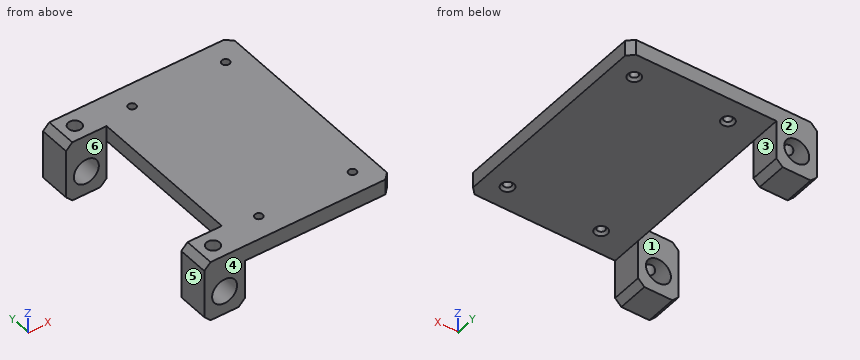
```python
from build123d import *

# Parameters (mm, degrees)
BOSS_EXTRUDE1_DEPTH   = 70
SKETCH2_R             = 0.75
CUT_EXTRUDE1_DEPTH    = 10
SKETCH3_W             = 25
SKETCH3_H             = 50
CUT_EXTRUDE2_DEPTH    = 13
SKETCH4_R             = 4
CUT_EXTRUDE3_DEPTH    = 96.524865873
SKETCH5_W             = 13
SKETCH5_H             = 50
BOSS_EXTRUDE2_DEPTH   = 5
SKETCH9_W             = 13
SKETCH9_H             = 5.5
CUT_EXTRUDE6_DEPTH    = 71
LPATTERN1_COUNT       = 2
LPATTERN1_PITCH       = 30
SKETCH10_W            = 13
SKETCH10_H            = 50
CUT_EXTRUDE7_DEPTH    = 95.235078394
CHAMFER1_SIZE         = 2
CHAMFER2_SIZE         = 2
M3_TAPPED_HOLE1_D     = 2.5
M3_TAPPED_HOLE1_DEPTH = 7.5
M3_TAPPED_HOLE1_TIP   = 0.751075774
M5_TAPPED_HOLE1_D     = 4.2
M5_TAPPED_HOLE1_DEPTH = 12.4
M5_TAPPED_HOLE1_TIP   = 1.2618073
M5_TAPPED_HOLE2_D     = 4.2
M5_TAPPED_HOLE2_DEPTH = 12.4
M5_TAPPED_HOLE2_TIP   = 1.2618073
CHAMFER3_SIZE         = 0.8


with BuildPart() as part:
    # Sketch1 → Boss-Extrude1 (new body)
    with BuildSketch(Plane(origin=(0, 0, 0), x_dir=(1, 0, 0), z_dir=(0, 1, 0))):
        Polygon((0, 0), (60, 0), (60, 5), (13, 5), (13, 25), (0, 25), align=None)
    extrude(amount=BOSS_EXTRUDE1_DEPTH)

    # Sketch2 → Cut-Extrude1 (cut)
    with BuildSketch(Plane.XY):
        with Locations((53, 62.5)):
            Circle(SKETCH2_R)
        with Locations((53, 7.5)):
            Circle(SKETCH2_R)
    cut_extrude1 = extrude(amount=-CUT_EXTRUDE1_DEPTH, mode=Mode.SUBTRACT)

    # Sketch3 → Cut-Extrude2 (cut)
    with BuildSketch(Plane.ZY):
        with Locations((-12.5, 35)):
            Rectangle(SKETCH3_W, SKETCH3_H)
    extrude(amount=-CUT_EXTRUDE2_DEPTH, mode=Mode.SUBTRACT)

    # Sketch4 → Cut-Extrude3 (cut, through all)
    with BuildSketch(Plane(origin=(0, 70, 0), x_dir=(1, 0, 0), z_dir=(0, 1, 0))):
        with Locations(Location((6.5, 12, 0), (0, 0, 270))):
            Circle(SKETCH4_R)
    extrude(amount=-CUT_EXTRUDE3_DEPTH, mode=Mode.SUBTRACT)

    # Sketch5 → Boss-Extrude2 (add)
    with BuildSketch(Plane.XY):
        with Locations((6.5, 35)):
            Rectangle(SKETCH5_W, SKETCH5_H)
    extrude(amount=-BOSS_EXTRUDE2_DEPTH)

    # Sketch9 → Cut-Extrude6 (cut)
    with BuildSketch(Plane(origin=(0, 70, 0), x_dir=(1, 0, 0), z_dir=(0, 1, 0))):
        with Locations((6.5, 22.25)):
            Rectangle(SKETCH9_W, SKETCH9_H)
    extrude(amount=-CUT_EXTRUDE6_DEPTH, mode=Mode.SUBTRACT)

    # LPattern1: Cut-Extrude1 ×2
    with Locations(*[(-i * LPATTERN1_PITCH, 0, 0) for i in range(1, LPATTERN1_COUNT)]):
        add(cut_extrude1, mode=Mode.SUBTRACT)

    # Sketch10 → Cut-Extrude7 (cut, through all)
    with BuildSketch(Plane(origin=(0, 0, -19.5), x_dir=(-1, 0, 0), z_dir=(0, 0, -1))):
        with Locations((-6.5, 35)):
            Rectangle(SKETCH10_W, SKETCH10_H)
    extrude(amount=-CUT_EXTRUDE7_DEPTH, mode=Mode.SUBTRACT)

    # Chamfer1
    chamfer1_edges = [part.edges().sort_by_distance(p)[0] for p in [
        (0, 65, 0),
        (0, 5, 0),
        (0, 5, -19.5),
        (0, 65, -19.5),
        (13, 5, -19.5),
        (13, 65, -19.5),
    ]]
    chamfer(chamfer1_edges, length=CHAMFER1_SIZE)

    # Chamfer2
    chamfer2_edges = [part.edges().sort_by_distance(p)[0] for p in [
        (60, 70, -2.5),
        (60, 0, -2.5),
    ]]
    chamfer(chamfer2_edges, length=CHAMFER2_SIZE)

    # M3 Tapped Hole1
    with Locations(Plane(origin=(23, 7.5, -5), x_dir=(-1, 0, 0), z_dir=(0, 0, -1))):
        with Locations((0, 0), (-30, 0), (-30, 55), (0, 55)):
            Hole(M3_TAPPED_HOLE1_D / 2, depth=M3_TAPPED_HOLE1_DEPTH)
            with Locations((0, 0, -(M3_TAPPED_HOLE1_DEPTH + M3_TAPPED_HOLE1_TIP / 2))):  # 118° drill point
                Cone(0, M3_TAPPED_HOLE1_D / 2, M3_TAPPED_HOLE1_TIP, mode=Mode.SUBTRACT)

    # M5 Tapped Hole1
    with Locations(Plane(origin=(6.5, 5, 0), x_dir=(1, 0, 0), z_dir=(0, 0, 1))):
        with Locations((0, 0)):
            Hole(M5_TAPPED_HOLE1_D / 2, depth=M5_TAPPED_HOLE1_DEPTH)
            with Locations((0, 0, -(M5_TAPPED_HOLE1_DEPTH + M5_TAPPED_HOLE1_TIP / 2))):  # 118° drill point
                Cone(0, M5_TAPPED_HOLE1_D / 2, M5_TAPPED_HOLE1_TIP, mode=Mode.SUBTRACT)

    # M5 Tapped Hole2
    with Locations(Plane(origin=(6.5, 65, 0), x_dir=(1, 0, 0), z_dir=(0, 0, 1))):
        with Locations((0, 0)):
            Hole(M5_TAPPED_HOLE2_D / 2, depth=M5_TAPPED_HOLE2_DEPTH)
            with Locations((0, 0, -(M5_TAPPED_HOLE2_DEPTH + M5_TAPPED_HOLE2_TIP / 2))):  # 118° drill point
                Cone(0, M5_TAPPED_HOLE2_D / 2, M5_TAPPED_HOLE2_TIP, mode=Mode.SUBTRACT)

    # Chamfer3
    chamfer3_edges = [part.edges().sort_by_distance(p)[0] for p in [
        (21.75, 62.5, -5),
        (51.75, 62.5, -5),
        (51.75, 7.5, -5),
        (21.75, 7.5, -5),
    ]]
    chamfer(chamfer3_edges, length=CHAMFER3_SIZE)


solid = part.part
```
Geometry: final body of the model. Coordinates: model frame, mm. Face numbers are marked on the shaded views. A direction names the side the tool comes from. Give positions to 0.01 mm unless a question says otherwise; leave off trailing zeros. Order: outer loops, then holes, each group sorted by start corner. A loop starts at its lowest first (then second) coordinate and runs counter-clockwise, first axis right, second up. Notation, with made-up numbers: M -13,24.5 L 15,24.5 A21 ccw 15,54.5 Z; hole C 51.5,-7.5 d11. An arc over 180 degrees is marked long. Answer as CSV lines item,"result". Start each with the question number.
1) Line query: line 1 (Y direction, x = 6.5, z = -2.5); line 2 (Y direction, x = 23, z = -1.6); line 3 (X direction, y = 5, z = -3.25). Output: solid intervals per line, ascending. Write a range as from..to.
2) Cut plane C-C (x = 6.5). Output: boundary loops of the cut face in (y, z).
3) Mould query, pull axis Y, two halves, no side actions, for the marked faces 4, 5 and 6. Classes: +Y half, -Y half, draft (parallel to the pull), parting line (faces both ways), or undercut.
4) First-contact query: P1, Ø14, axis at x = 36.5, y = 47, coming from the -Z side; P2, Ø3, axis at y = 3.5, z = -10.5, coming from the +X side; P3, Ø1.5, axis at x = 53, y = 62.5, coming from the +Z side; P4, Ø5.5, axis at y = 37, z = -2.5, coming from the -X side. Flat tips, straight axial feed; report the tip coordinate or a pass-through.
5) Set-up query: the marked faces 1, 2 and 3. Return all of +Z, -Z, +X, -X, +Y, -Y with unobstructed straight access to the full face (end or side cutting, diameter ignored); none if empty.
6) Cut plane A-A (x = 23). Output: boundary loops of the cut face in (y, z), then the cut area to 3 significant figures.
7) Cut plane B-B (z = -11.75). Output: boundary loops of the cut face in (x, y), then the cut area to 3 significant figures.
8) Cut plane D-D (y = 13). Output: boundary loops of the cut face in (x, z), then the cut area to 3 significant figures.
Findings below:
1,line 1,"y = 0..2.9, 7.1..10, 60..62.9, 67.1..70"
1,line 2,"y = 0..6.25, 8.75..61.25, 63.75..70"
1,line 3,"x = 0..4.4, 8.6..60"
2,outline,"M 0,-19.5 L 10,-19.5 L 10,-16 L 0,-16 Z; M 0,-8 L 2.9,-8 L 2.9,0 L 0,0 Z; M 7.1,-8 L 10,-8 L 10,0 L 7.1,0 Z; M 60,-19.5 L 70,-19.5 L 70,-16 L 60,-16 Z; M 60,-8 L 62.9,-8 L 62.9,0 L 60,0 Z; M 67.1,-8 L 70,-8 L 70,0 L 67.1,0 Z"
3,face 4,"-Y half"
3,face 5,"draft"
3,face 6,"undercut"
4,P1,"stops at z = -5"
4,P2,"stops at x = 13"
4,P3,"passes through"
4,P4,"stops at x = 13"
5,face 1,"+Z, -Z, -X"
5,face 2,"+Z, -Z, +X, -X, +Y"
5,face 3,"-Z, +X, +Y, -Y"
6,outline,"M 0,-5 L 5.45,-5 L 6.25,-4.2 L 6.25,0 L 0,0 Z; M 8.75,-4.2 L 9.55,-5 L 60.45,-5 L 61.25,-4.2 L 61.25,0 L 8.75,0 Z; M 63.75,-4.2 L 64.55,-5 L 70,-5 L 70,0 L 63.75,0 Z"
6,area,"324 mm²"
7,outline,"M 0,0 L 2.51,0 L 2.51,10 L 0,10 Z; M 0,60 L 2.51,60 L 2.51,70 L 0,70 Z; M 10.49,0 L 13,0 L 13,10 L 10.49,10 Z; M 10.49,60 L 13,60 L 13,70 L 10.49,70 Z"
7,area,"100 mm²"
8,outline,"M 13,-5 L 60,-5 L 60,0 L 13,0 Z"
8,area,"235 mm²"
